Geometry check sheet. Reference: drawing and pictorial views, mm from the part's lowest x, y, z. Give positions to 0.01 mm unless a question says otherwise; leave off trailing zeros. Order: outer loops, then holes, each group sorted by start corner. A loop starts at its lowest first (then second) coordinate and runs counter-clockwise, first axis right, second up. Notation, with made-up numbers: M 48,-38.5 L 55,-38.5 A29 cw 55,-11.5 Z; hole C -36.75,2.25 d8. An arc over 180 degrees is marked long. Answer as CSV lines item,"result". Start each with the question number.
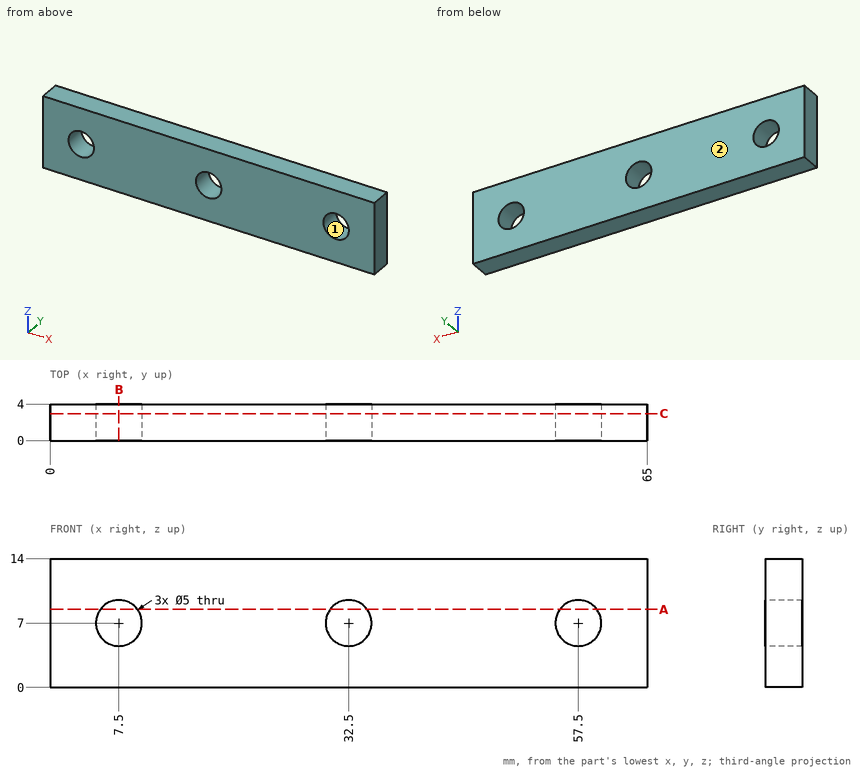
Item 1: Section check B-B on x = 7.5. Record the boundary of the cut face in (y, z), then the cut area to 3 significant figures.
Item 2: Scan lines: line 1 along X through (y, z) = (3.55, 7.25); line 2 along Z through (x, y) = (57.5, 1.55); line 3 along X through (y, z) = (1.9, 7.75). Record each from-to range of solid material in increasing order.
Item 3: Draft check along X on the marked faces 1 and 2. Enter one of: pulls with the +X half, pulls with the -X half, needs draft (parallel to the pull), parting line crosses it, or undercut.
Item 4: Section check A-A on z = 8.5. Record the boundary of the cut face in (x, y).
Item 5: Section check C-C on y = 2.95. Record the boundary of the cut face in (x, z), then the cut area to 3 significant figures.
Numbers:
1,outline,"M 0,0 L 4,0 L 4,4.5 L 0,4.5 Z; M 0,9.5 L 4,9.5 L 4,14 L 0,14 Z"
1,area,"36.0 mm2"
2,line 1,"0 to 5.01, 9.99 to 30.01, 34.99 to 55.01, 59.99 to 65"
2,line 2,"0 to 4.5, 9.5 to 14"
2,line 3,"0 to 5.12, 9.88 to 30.12, 34.88 to 55.12, 59.88 to 65"
3,face 1,"undercut"
3,face 2,"needs draft"
4,outline,"M 0,0 L 5.5,0 L 5.5,4 L 0,4 Z; M 9.5,0 L 30.5,0 L 30.5,4 L 9.5,4 Z; M 34.5,0 L 55.5,0 L 55.5,4 L 34.5,4 Z; M 59.5,0 L 65,0 L 65,4 L 59.5,4 Z"
5,outline,"M 0,0 L 65,0 L 65,14 L 0,14 Z; hole C 7.5,7 d5; hole C 32.5,7 d5; hole C 57.5,7 d5"
5,area,"851 mm2"
